```python
from build123d import *

# Parameters (mm, degrees)
SKETCH_1_W          = 300
SKETCH_1_H          = 180
EXTRUDE_1_DEPTH     = 14
SKETCH_2_W          = 42
SKETCH_2_H          = 180
CUT_EXTRUDE_1_DEPTH = 1.5
CUT_EXTRUDE_2_REACH = 177.488
SKETCH_3_R          = 32.5


with BuildPart() as part:
    # 草图1 → 凸台-拉伸1 (new body)
    with BuildSketch(Plane.XY):
        Rectangle(SKETCH_1_W, SKETCH_1_H)
    extrude(amount=EXTRUDE_1_DEPTH)

    # 草图2 → 切除-拉伸1 (cut)
    with BuildSketch(Plane(origin=(0, 0, 0), x_dir=(-1, 0, 0), z_dir=(0, 0, -1))):
        with Locations((129, 0)):
            Rectangle(SKETCH_2_W, SKETCH_2_H)
        with Locations((-129, 0)):
            Rectangle(SKETCH_2_W, SKETCH_2_H)
    extrude(amount=-CUT_EXTRUDE_1_DEPTH, mode=Mode.SUBTRACT)

    # 草图3 → 切除-拉伸2 (cut, up to next)
    with BuildSketch(Plane.XY.offset(14), mode=Mode.PRIVATE) as cut_extrude_2_sk1:
        Circle(SKETCH_3_R)
    cut_extrude_2_tool1 = extrude(cut_extrude_2_sk1.sketch, amount=-CUT_EXTRUDE_2_REACH, mode=Mode.PRIVATE) & part.part
    add(cut_extrude_2_tool1.solids().sort_by_distance((0, 0, 14))[0], mode=Mode.SUBTRACT)


solid = part.part
```
Read the model definition and answer for the solid it produces. Units are mm, in the model's axes. A direction names the side the tool comes from. Give positions to 0.01 mm unless a question says otherwise; leave off trailing zeros. Write each loop counter-clockwise with the first axis right and the second up, starting at its lowest first coordinate (ties: lowest second). Pieces come first, ordered by that corner, then holes. Notation, with made-up numbers: (31.5, 80) - (82.5, 80) arc R37 cw to (82.5, 116) - close; hole circle Ø5 at (13, 74). An arc over 180 degrees is marked (long way). Write item = value, one per line. Start each with the question number.
Item 1: A tool of negligible diameter and unlimited length cuts with its end or side. For faces 1 (the flat face through (-26, 21, 0)), 2 (the flat face through (129, 1, 1.5)), 3 (the flat face through (-129, 1, 1.5)), from which of +Z, -Z, +X, -X, +Y, -Y can it reach the whole face along a straight path? Write none if from no direction.
Item 2: Find section C-C (x = 0). Give the vertices of the cut face in (y, z), then the cut area to 3 significant figures.
Item 3: Find section A-A (y = 0). Give the vertices of the cut face in (x, z), then the cut area to 3 significant figures.
Item 4: Find the intervals of material crossed by probe 1 along Y at (x, z) = (0, 6.75); probe 2 along Z at (x, y) = (125.5, -5); probe 3 along Y at (x, z) = (26.5, 7), in increasing order. Write a range as [from, to].
Item 5: Find section D-D (y = -38.5). Give the vertices of the cut face in (x, z).
Item 6: The mould has two halves that part along Y. Classify faces 4 (the flat face through (150, -1, 8)), 5 (the cylindrical face through (31, 9.76, 7.1)), 6 (the flat face through (-2, -90, 7)): +Y half, -Y half, draft (parallel to the pull), parting line (faces both ways), or undercut.
Item 7: Find section B-B (z = 4). Give the vertices of the cut face in (x, y), then the cut area to 3 significant figures.
Item 8: Each of these flat-tipped pins is pushed along its axis until it touches: P1, Ø8, axis at x = -103.5, y = 14.5, coming from the -Z side; P2, Ø0.8, axis at y = -2, z = 1, coming from the +X side; P3, Ø12.5, axis at x = -124, y = -5, coming from the -Z side. Where does it stop, or does it pass through?
Response:
q1.face_1 = -Z, +X, -X, +Y, -Y
q1.face_2 = -Z, +X, +Y, -Y
q1.face_3 = -Z, -X, +Y, -Y
q2.outline = (-90, 0) - (-32.5, 0) - (-32.5, 14) - (-90, 14) - close; (32.5, 0) - (90, 0) - (90, 14) - (32.5, 14) - close
q2.area = 1,610 mm²
q3.outline = (-150, 1.5) - (-108, 1.5) - (-108, 0) - (-32.5, 0) - (-32.5, 14) - (-150, 14) - close; (32.5, 0) - (108, 0) - (108, 1.5) - (150, 1.5) - (150, 14) - (32.5, 14) - close
q3.area = 3,160 mm²
q4.probe_1 = [-90, -32.5], [32.5, 90]
q4.probe_2 = [1.5, 14]
q4.probe_3 = [-90, -18.81], [18.81, 90]
q5.outline = (-150, 1.5) - (-108, 1.5) - (-108, 0) - (108, 0) - (108, 1.5) - (150, 1.5) - (150, 14) - (-150, 14) - close
q6.face_4 = draft
q6.face_5 = undercut
q6.face_6 = -Y half
q7.outline = (-150, -90) - (150, -90) - (150, 90) - (-150, 90) - close; hole circle Ø65 at (0, 0)
q7.area = 50,700 mm²
q8.P1 = 0
q8.P2 = 108
q8.P3 = 1.5
